```python
from build123d import *

# Parameters (mm, degrees)
COLD_FORMED_SQUARE_HOLLOW_SECTION_GB_T_6_DEPTH = 390


with BuildPart() as part:
    # Sketch1 → Cold-formed square hollow section GB/T 6728-2002 50 X 50 X 4(1) (new body)
    with BuildSketch(Plane.YZ.offset(-88.434077868)):
        with BuildLine():
            Line((-17, -25), (17, -25))
            ThreePointArc((17, -25), (22.656854249, -22.656854249), (25, -17))
            Line((25, -17), (25, 17))
            ThreePointArc((25, 17), (22.656854249, 22.656854249), (17, 25))
            Line((17, 25), (-17, 25))
            ThreePointArc((-17, 25), (-22.656854249, 22.656854249), (-25, 17))
            Line((-25, 17), (-25, -17))
            ThreePointArc((-25, -17), (-22.656854249, -22.656854249), (-17, -25))
        make_face()
        with BuildLine():
            Line((-17, -20), (17, -20))
            ThreePointArc((17, -20), (19.121320344, -19.121320344), (20, -17))
            Line((20, -17), (20, 17))
            ThreePointArc((20, 17), (19.121320344, 19.121320344), (17, 20))
            Line((17, 20), (-17, 20))
            ThreePointArc((-17, 20), (-19.121320344, 19.121320344), (-20, 17))
            Line((-20, 17), (-20, -17))
            ThreePointArc((-20, -17), (-19.121320344, -19.121320344), (-17, -20))
        make_face(mode=Mode.SUBTRACT)
    extrude(amount=COLD_FORMED_SQUARE_HOLLOW_SECTION_GB_T_6_DEPTH)


solid = part.part
```
Geometry check sheet. Reference: the model listing, model coordinates, mm. A direction names the side the tool comes from. Round coordinates to 2 decimals unless told otherwise and drop trailing zeros. Loops run counter-clockwise (first coordinate to the right, second up) from the corner with the lowest first, then second, coordinate; pieces in that order, holes last. Notation, with made-up numbers: (73.5, 16.25) - (129.5, 16.25) arc R16 ccw to (129.5, 47.25) - close; hole circle Ø8 at (2, -15.5). An arc over 180 degrees is marked (long way). Write item = value, one per line. Start each with the question number.
1. Mould release check, pull along Z, two halves, no side actions. Record for faces 3 (the face through (103.836, 22.719, 22.594)), 4 (the face through (-88.434, -23, 0)), 5 (the face through (104, 0, -20)): released by +Z, released by -Z, zero draft, split by the parting line, or undercut.
2. Section check C-C on x = -36. Enter the section's corners in (y, z).
3. Section check A-A on y = -13. Enter the section's corners in (x, z).
4. Thickness scan on line 1 (Z direction, x = -38.5, y = -12); line 2 (Z direction, x = 118, y = -19.5). Record the ranges inside material, lowest first.
5. Set-up check for faces 1 (the face through (104, 20, 0)), 2 (the face through (103.836, -22.594, 22.719)): record each of +Z, -Z, +X, -X, +Y, -Y from which the full face is reachable in a straight line by a thin tool's end or side.
Working result:
q1.face_3 = released by +Z
q1.face_4 = zero draft
q1.face_5 = undercut
q2.outline = (-25, -17) arc R8 ccw to (-17, -25) - (17, -25) arc R8 ccw to (25, -17) - (25, 17) arc R8 ccw to (17, 25) - (-17, 25) arc R8 ccw to (-25, 17) - close; hole (-20, -17) arc R3 ccw to (-17, -20) - (17, -20) arc R3 ccw to (20, -17) - (20, 17) arc R3 ccw to (17, 20) - (-17, 20) arc R3 ccw to (-20, 17) - close
q3.outline = (-88.43, -25) - (301.57, -25) - (301.57, -20) - (-88.43, -20) - close; (-88.43, 20) - (301.57, 20) - (301.57, 25) - (-88.43, 25) - close
q4.line_1 = -25 to -20, 20 to 25
q4.line_2 = -24.6 to -18.66, 18.66 to 24.6
q5.face_1 = +X, -X
q5.face_2 = +Z, +X, -X, -Y
